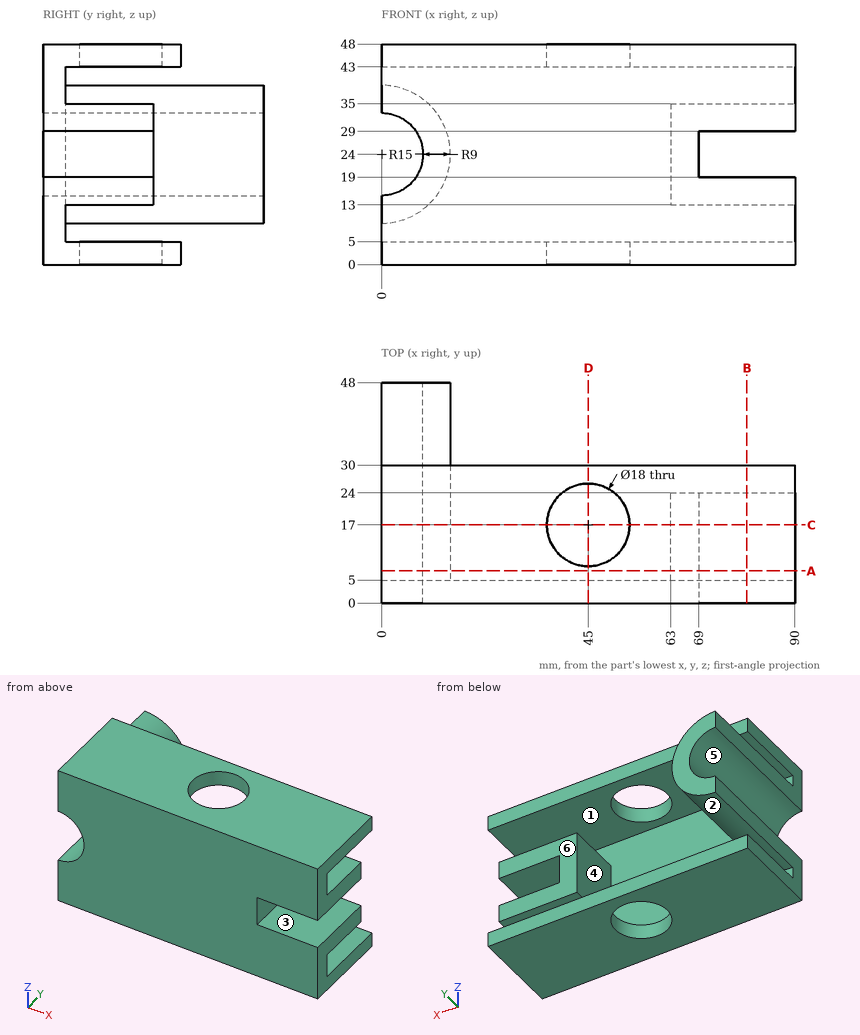
Geometry: see drawing. Coordinates: mm, zero at the bounding-box minimum. A direction names the side the tool comes from. Give positions to 0.01 mm unless a question says otherwise; leave off trailing zeros. Loops run counter-clockwise (first coordinate to the right, second up) from the corner with the lowest first, then second, coordinate; pieces in that order, holes last. Notation, with made-up numbers: (18, 51) -> (36, 51) arc R21 ccw to (36, 58) -> close; hole circle Ø6 at (-29, 69). An arc over 180 degrees is marked (long way). Use CSV: the item, a comma, the result in double quotes.
(1) Cut plane B-B (x = 79.5). Output: boundary loops of the cut face in (y, z).
From the geometry:
outline,"(0, 0) -> (30, 0) -> (30, 5) -> (5, 5) -> (5, 13) -> (24, 13) -> (24, 19) -> (0, 19) -> close; (0, 29) -> (24, 29) -> (24, 35) -> (5, 35) -> (5, 43) -> (30, 43) -> (30, 48) -> (0, 48) -> close"
(2) Pull-direction query (X, two-part tool) for the marked faces 4, 5 and 6; classes: released by +X, released by -X, zero draft, split by the parting line, or undercut.
From the geometry:
face 4,"undercut"
face 5,"released by -X"
face 6,"zero draft"
(3) First-contact query: P1, Ø24, axis at x = 82, z = 23.5, coming from the +Y side; P2, Ø9.5, axis at y = 10.5, z = 23.5, coming from the -X side; P3, Ø4, axis at x = 32, z = 2.5, coming from the +Y side; P4, Ø11, axis at x = 45, y = 17, coming from the +Z side. Flat tips, straight axial feed; report the tip coordinate or a pass-through.
From the geometry:
P1,"y = 24"
P2,"x = 7.31"
P3,"y = 30"
P4,"through"
(4) Access query for the marked faces 1, 2 and 3. Directions: +Z, -Z, +X, -X, +Y, -Y. A direction counts if a zero-diameter tool reaches every point of the face in a straight line with its end or side. Return the directions, or none.
From the geometry:
face 1,"+X, -X, +Y"
face 2,"+Y"
face 3,"+X, +Y, -Y"
(5) Cut plane C-C (y = 17). Output: boundary loops of the cut face in (x, z), plus the area to 3 significant figures.
From the geometry:
outline,"(0, 0) -> (36, 0) -> (36, 5) -> (0, 5) -> close; (0, 9) arc R15 ccw to (0, 39) -> (0, 33) arc R9 cw to (0, 15) -> close; (0, 43) -> (36, 43) -> (36, 48) -> (0, 48) -> close; (54, 0) -> (90, 0) -> (90, 5) -> (54, 5) -> close; (54, 43) -> (90, 43) -> (90, 48) -> (54, 48) -> close; (63, 13) -> (90, 13) -> (90, 19) -> (69, 19) -> (69, 29) -> (90, 29) -> (90, 35) -> (63, 35) -> close"
area,"1,330 mm^2"
(6) Cut plane D-D (x = 45). Output: boundary loops of the cut face in (y, z), plus the area to 3 significant figures.
From the geometry:
outline,"(0, 0) -> (8, 0) -> (8, 5) -> (5, 5) -> (5, 43) -> (8, 43) -> (8, 48) -> (0, 48) -> close; (26, 0) -> (30, 0) -> (30, 5) -> (26, 5) -> close; (26, 43) -> (30, 43) -> (30, 48) -> (26, 48) -> close"
area,"310 mm^2"
(7) Ray query, line 1 along Z through (x, y) = (67.5, 19); line 2 along Y through (x, z) = (45, 44.8); line 3 along Z through (x, y) = (18, 24). Return the intervals inside material, ascending. Write a range as [from, to].
From the geometry:
line 1,"[0, 5], [13, 35], [43, 48]"
line 2,"[0, 8], [26, 30]"
line 3,"[0, 5], [43, 48]"
(8) Cut plane A-A (y = 7). Output: boundary loops of the cut face in (x, z).
From the geometry:
outline,"(0, 0) -> (90, 0) -> (90, 5) -> (0, 5) -> close; (0, 9) arc R15 ccw to (0, 39) -> (0, 33) arc R9 cw to (0, 15) -> close; (0, 43) -> (90, 43) -> (90, 48) -> (0, 48) -> close; (63, 13) -> (90, 13) -> (90, 19) -> (69, 19) -> (69, 29) -> (90, 29) -> (90, 35) -> (63, 35) -> close"
